```python
from build123d import *

# Parameters (mm, degrees)
SKETCH1_R           = 33
SKETCH1_R_2         = 9
BOSS_EXTRUDE1_DEPTH = 40
CHAMFER2_SIZE       = 180
CHAMFER2_SIZE2      = 120
CHAMFER3_SIZE       = 160
M24_TAPPED_HOLE1_D  = 21
FILLET1_R           = 15
CUT_EXTRUDE1_DEPTH  = 1446.060552365
FILLET2_R           = 10
FILLET3_R           = 10


with BuildPart() as part:
    # Sketch1 → Boss-Extrude1 (new body)
    with BuildSketch(Plane.XY):
        Polygon((1240, 420), (1240, 650), (1290, 650), (1290, 0), (0, 0), (0, 420), align=None)
        with Locations((205, 360)):
            Circle(SKETCH1_R, mode=Mode.SUBTRACT)
        with Locations((1269, 405)):
            Circle(SKETCH1_R_2, mode=Mode.SUBTRACT)
        with Locations((1269, 605)):
            Circle(SKETCH1_R_2, mode=Mode.SUBTRACT)
    extrude(amount=BOSS_EXTRUDE1_DEPTH)

    # Chamfer2
    chamfer2_edges = [part.edges().sort_by_distance(p)[0] for p in [
        (0, 420, 20),
    ]]
    chamfer2_side = [part.faces().sort_by_distance(p)[0] for p in [
        (620, 420, 20),
    ]]
    chamfer(chamfer2_edges, length=CHAMFER2_SIZE, length2=CHAMFER2_SIZE2, reference=chamfer2_side[0])

    # Chamfer3
    chamfer3_edges = [part.edges().sort_by_distance(p)[0] for p in [
        (0, 0, 20),
    ]]
    chamfer(chamfer3_edges, length=CHAMFER3_SIZE)

    # M24 Tapped Hole1 (through all)
    with Locations(Plane(origin=(540, 150, 40), x_dir=(1, 0, 0), z_dir=(0, 0, 1))):
        with Locations((0, 0), (620, 0), (-244.064633972, 118.316259911)):
            Hole(M24_TAPPED_HOLE1_D / 2)

    # Fillet1
    fillet1_edges = [part.edges().sort_by_distance(p)[0] for p in [
        (1240, 420, 20),
        (1240, 650, 20),
    ]]
    fillet(fillet1_edges, radius=FILLET1_R)

    # Sketch2 → Cut-Extrude1 (cut, through all)
    with BuildSketch(Plane.XY.offset(40)):
        Polygon((585, 0), (735, 0), (700, 80), (620, 80), align=None)
        Polygon((975, 0), (1125, 0), (1090, 80), (1010, 80), align=None)
    extrude(amount=-CUT_EXTRUDE1_DEPTH, mode=Mode.SUBTRACT)

    # Fillet2
    fillet2_edges = [part.edges().sort_by_distance(p)[0] for p in [
        (700, 80, 20),
        (735, 0, 20),
        (585, 0, 20),
        (620, 80, 20),
        (1010, 80, 20),
        (1090, 80, 20),
        (1125, 0, 20),
        (975, 0, 20),
    ]]
    fillet(fillet2_edges, radius=FILLET2_R)

    # Fillet3
    fillet3_edges = [part.edges().sort_by_distance(p)[0] for p in [
        (0, 300, 20),
        (180, 420, 20),
        (160, 0, 20),
        (0, 160, 20),
    ]]
    fillet(fillet3_edges, radius=FILLET3_R)


solid = part.part
```
Design review of the part built by this model. Coordinates are the model's own, in mm. A direction names the side the tool comes from. Coordinates: 2 decimals unless noted, no trailing zeros. Order: outer loops, then holes, each group sorted by start corner. A loop starts at its lowest first (then second) coordinate and runs counter-clockwise, first axis right, second up. Notation, with made-up numbers: (64.25, 7.25) - (99.25, 7.25) arc R28 cw to (99.25, 36.25) - close; hole circle Ø8 at (46, 33). An arc over 180 degrees is marked (long way). One line per question, with ' | ' between items.
Q1. For faces 1 (the flat face through (697, 420, 20)), 2 (the flat face through (1107.71, 39.52, 20.28)), 3 (the flat face through (1212, 0, 20)), list the 3-axis set-ups (+Z, -Z, +X, -X, +Y, -Y) from which the entire face can be reached by the end or side of a thin tool; tool diameter is ignored.
Answer key:
face 1: +Z, -Z, -X, +Y | face 2: +Z, -Z, -Y | face 3: +Z, -Z, +X, -X, -Y
Q2. To check wall thickness, follow line 1 along Y through (x, z) = (1269, 22); line 2 along Y through (x, z) = (540, 31); line 3 along Y through (x, z) = (205, 10). State the ranges of each line that lie inside material, in increasing order.
Answer key:
line 1: y = 0 to 396, 414 to 596, 614 to 650 | line 2: y = 0 to 139.5, 160.5 to 420 | line 3: y = 0 to 327, 393 to 420
Q3. Consider section D-D, the plane x = 905. Give the boundary of the cut face in (y, z).
Answer key:
outline: (0, 0) - (420, 0) - (420, 40) - (0, 40) - close
Q4. Consider section B-B, the plane x = 205. Give the boundary of the cut face in (y, z).
Answer key:
outline: (0, 0) - (327, 0) - (327, 40) - (0, 40) - close; (393, 0) - (420, 0) - (420, 40) - (393, 40) - close
Q5. Consider section A-A, the plane y = 360. Give the boundary of the cut face in (x, z).
Answer key:
outline: (90, 0) - (172, 0) - (172, 40) - (90, 40) - close; (238, 0) - (1290, 0) - (1290, 40) - (238, 40) - close
Q6. The part is to be moulded in two halves that separate along X. For faces 4 (the flat face through (654, 257, 0)), 5 (the flat face through (1290, 330, 20)), 6 (the flat face through (1240, 534, 20)), 7 (the flat face through (992.71, 40.48, 20.28)), say which applies: +X half, -X half, draft (parallel to the pull), parting line (faces both ways), or undercut.
Answer key:
face 4: draft | face 5: +X half | face 6: -X half | face 7: undercut
Q7. Clearance check with flat-ended pins moving along their axes: pin 1 Ø4 at (x, z) = (1072.5, 14.5) entering from +Y; pin 2 Ø1 at (x, y) = (788, 221) entering from -Z. State where each tip first meets the part, or that it passes through.
Answer key:
pin 1: stops at y = 420 | pin 2: stops at z = 0
Q8. Consider section C-C, the plane z = 14. Give the number of separate pieces and of enclosed holes in the cut face, then the cut area to 3 significant figures.
Answer key:
separate pieces: 1 | enclosed holes: 6 | area: 506,000 mm2
